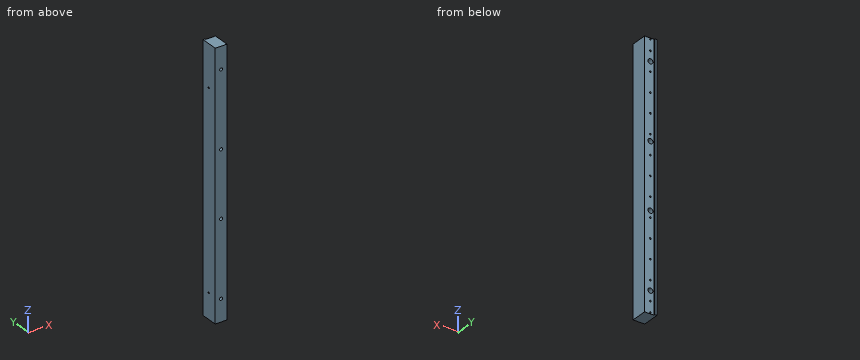
```python
from build123d import *

# Parameters (mm, degrees)
EXTRUDE_1_DEPTH           = 397
HOLE_WIZARD_M6_1_D        = 5
HOLE_WIZARD_M6_1_DEPTH    = 15
HOLE_WIZARD_M6_1_TIP      = 1.502151548
PATTERN_LINEAR_1_COUNT    = 13
PATTERN_LINEAR_1_PITCH    = 60
HOLE_WIZARD_1_D           = 9
HOLE_WIZARD_1_CBORE_D     = 15
HOLE_WIZARD_1_CBORE_DEPTH = 15
HOLE_WIZARD_M5_1_D        = 4.2
HOLE_WIZARD_M5_1_DEPTH    = 12.4
HOLE_WIZARD_M5_1_TIP      = 1.2618073


with BuildPart() as part:
    # 草图1 → 凸台-拉伸1 (new, symmetric)
    with BuildSketch(Plane.XY):
        Polygon((0, 0), (36, 0), (36, 50.5), (6.5, 50.5), (6.5, 53.5), (0, 53.5), align=None)
    extrude(amount=EXTRUDE_1_DEPTH, both=True)

    # M6 螺纹孔1
    with Locations(Plane.ZY):
        with Locations((-320, 28.5), (270, 28.5)):
            Hole(HOLE_WIZARD_M6_1_D / 2, depth=HOLE_WIZARD_M6_1_DEPTH)
            with Locations((0, 0, -(HOLE_WIZARD_M6_1_DEPTH + HOLE_WIZARD_M6_1_TIP / 2))):  # 118° drill point
                Cone(0, HOLE_WIZARD_M6_1_D / 2, HOLE_WIZARD_M6_1_TIP, mode=Mode.SUBTRACT)

    # 草图4 → M6 螺纹孔2 (revolve, cut)
    with BuildSketch(Plane(origin=(18, 50.5, -360), x_dir=(0, 0, 1), z_dir=(1, 0, 0))):
        Polygon((0, 0), (0, 16.502151548), (2.5, 15), (2.5, 0), align=None)
    hole_wizard_m6_2 = revolve(axis=Axis((18, 56.85, -360), (0, -1, 0)), mode=Mode.SUBTRACT)

    # 阵列(线性)1: M6 螺纹孔2 ×13
    with Locations(*[(0, 0, i * PATTERN_LINEAR_1_PITCH) for i in range(1, PATTERN_LINEAR_1_COUNT)]):
        add(hole_wizard_m6_2, mode=Mode.SUBTRACT)

    # 打孔尺寸(%根据)内六角圆柱头螺钉的类型1 (through all)
    with Locations(Plane(origin=(0, 50.5, 0), x_dir=(1, 0, 0), z_dir=(0, 1, 0))):
        with Locations((18, 330), (18, 100), (18, -100), (18, -330)):
            CounterBoreHole(HOLE_WIZARD_1_D / 2, HOLE_WIZARD_1_CBORE_D / 2, HOLE_WIZARD_1_CBORE_DEPTH)

    # M5 螺纹孔1
    with Locations(Plane(origin=(0, 50.5, 0), x_dir=(1, 0, 0), z_dir=(0, 1, 0))):
        with Locations((18, 393), (18, -393)):
            Hole(HOLE_WIZARD_M5_1_D / 2, depth=HOLE_WIZARD_M5_1_DEPTH)
            with Locations((0, 0, -(HOLE_WIZARD_M5_1_DEPTH + HOLE_WIZARD_M5_1_TIP / 2))):  # 118° drill point
                Cone(0, HOLE_WIZARD_M5_1_D / 2, HOLE_WIZARD_M5_1_TIP, mode=Mode.SUBTRACT)


solid = part.part
```
The listing builds one solid part. Answer for the finished solid, in the listing's coordinates (mm). Round coordinates to 2 decimals unless told otherwise and drop trailing zeros. Loops run counter-clockwise (first coordinate to the right, second up) from the corner with the lowest first, then second, coordinate; pieces in that order, holes last.
1) Given P1, Ø16.5, axis at x = 16.5, z = 100.5, coming from the +Y side; P2, Ø7.5, axis at x = 15.5, z = -101, coming from the +Y side; P3, Ø4, axis at x = 18, z = -300, coming from the +Y side; P4, Ø5.5, axis at x = 18, z = -100, coming from the -Y side, each flat-ended and moving along its own axis, determine where each tip first touches the part or whether it passes through.
Outcome:
P1: stops at y = 50.5
P2: stops at y = 35.5
P3: stops at y = 35.2
P4: passes through
2) Consider line 1 (X direction, y = 46, z = 100); line 2 (Z direction, x = 19, y = 4.5); line 3 (X direction, y = 27, z = -330). Determine where each line is inside the solid, lowest interval first.
Outcome:
line 1: x = 0 to 10.5, 25.5 to 36
line 2: z = -397 to -334.39, -325.61 to -104.39, -95.61 to 95.61, 104.39 to 325.61, 334.39 to 397
line 3: x = 0 to 13.5, 22.5 to 36
3) A cutting plane is placed at A-A on z = 19. Determine the outline of the cut face in (x, y), plus the area to 3 significant figures.
Outcome:
outline: (0, 0) - (36, 0) - (36, 50.5) - (6.5, 50.5) - (6.5, 53.5) - (0, 53.5) - close
area: 1,840 mm2
